CAD build for the part. Positions are in the model's coordinates, mm. A direction names the side the tool comes from. Coordinates: 2 decimals unless noted, no trailing zeros. Order: outer loops, then holes, each group sorted by start corner. A loop starts at its lowest first (then second) coordinate and runs counter-clockwise, first axis right, second up. Notation, with made-up numbers: (-20, 79) - (1, 79) arc R20 ccw to (1, 100) - close; hole circle Ø7 at (72, 74.25). An arc over 180 degrees is marked (long way). Return JSON: item names as keys, results as strings.
from build123d import *

# Parameters (mm, degrees)
EYE_PLATE_11MM_DEPTH    = 11
FLOOR_PLATE_11MM_DEPTH  = 11
SIDE_WALL_11MM_DEPTH    = 11
INCLINED_WEB_PROFILE_W  = 102
INCLINED_WEB_PROFILE_H  = 76
INCLINED_WEB_11MM_DEPTH = 11
END_CAP_PROFILE_W       = 35
END_CAP_PROFILE_H       = 76
END_CAP_16MM_DEPTH      = 16
PIVOT_BORE_PROFILE_R    = 19
PIVOT_BORE_38_DEPTH     = 11


with BuildPart() as part:
    # Eye Plate Profile → Eye Plate 11mm (new body)
    with BuildSketch(Plane.XY):
        with BuildLine():
            Line((0, 0), (113, 0))
            Line((113, 0), (113, 63))
            Line((113, 63), (25, 63))
            ThreePointArc((25, 63), (7.32233047, 55.67766953), (0, 38))
            Line((0, 38), (0, 0))
        make_face()
    extrude(amount=EYE_PLATE_11MM_DEPTH)

    # Floor Plate Profile → Floor Plate 11mm (add)
    with BuildSketch(Plane(origin=(113, 0, 0), x_dir=(0, 0, -1), z_dir=(1, 0, 0))):
        Polygon((0, 0), (76, 0), (76, 100), (0, 63), align=None)
    extrude(amount=-FLOOR_PLATE_11MM_DEPTH)

    # Side Wall Profile → Side Wall 11mm (add)
    with BuildSketch(Plane(origin=(0, 0, -76), x_dir=(-1, 0, 0), z_dir=(0, 0, -1))):
        Polygon((-113, 0), (0, 0), (0, 11), (-75, 100), (-113, 100), align=None)
    extrude(amount=SIDE_WALL_11MM_DEPTH)

    # Inclined Web Profile → Inclined Web 11mm (add)
    with BuildSketch(Plane.XZ):
        with Locations((51, -38)):
            Rectangle(INCLINED_WEB_PROFILE_W, INCLINED_WEB_PROFILE_H)
    extrude(amount=-INCLINED_WEB_11MM_DEPTH)

    # End Cap Profile → End Cap 16mm (add)
    with BuildSketch(Plane(origin=(0, 11, 0), x_dir=(1, 0, 0), z_dir=(0, 1, 0))):
        with Locations((84.5, 38)):
            Rectangle(END_CAP_PROFILE_W, END_CAP_PROFILE_H)
    extrude(amount=END_CAP_16MM_DEPTH)

    # Pivot Bore Profile → Pivot Bore Ø38 (cut)
    with BuildSketch(Plane.XY.offset(11)):
        with Locations((25, 38)):
            Circle(PIVOT_BORE_PROFILE_R)
    extrude(amount=-PIVOT_BORE_38_DEPTH, mode=Mode.SUBTRACT)


solid = part.part
Item 1: Band-saw the part on A-A, the plane x = 69. List the corners of the cut face in (y, z).
Findings below:
{"outline": "(0, -87) - (92.88, -87) - (92.88, -76) - (27, -76) - (27, 0) - (63, 0) - (63, 11) - (0, 11) - close"}
Item 2: Band-saw the part on D-D, the plane x = 17. List the corners of the cut face in (y, z).
Findings below:
{"outline": "(0, -87) - (31.17, -87) - (31.17, -76) - (11, -76) - (11, 0) - (20.77, 0) - (20.77, 11) - (0, 11) - close; (55.23, 0) - (61.69, 0) - (61.69, 11) - (55.23, 11) - close"}
Item 3: Mould opens along Z. For faces 1 (the flat face through (107.58, 81.76, -38.53)), 2 (the flat face through (67, 19, -37)), 3 (the flat face through (56, 0, -37)) say: released by +Z, released by -Z, zero draft, split by the parting line, or undercut.
Findings below:
{"face 1": "released by +Z", "face 2": "undercut", "face 3": "zero draft"}
Item 4: Band-saw the part on B-B, the plane y = 30. List the corners of the cut face in (x, z).
Findings below:
{"outline": "(0, 0) - (7.77, 0) - (7.77, 11) - (0, 11) - close; (16.01, -87) - (113, -87) - (113, 11) - (42.23, 11) - (42.23, 0) - (102, 0) - (102, -76) - (16.01, -76) - close"}
Item 5: Wall check: L1, parallel to Z at x = 77, y = 39; L2, parallel to Y at x = 25, z = 8; L3, parallel to Y at x = 88, z = -18. Give the ranges that are in metal, low to high. Write a range as [from, to].
Findings below:
{"L1": "z = [-87, -76], [0, 11]", "L2": "y = [0, 19], [57, 63]", "L3": "y = [0, 27]"}
Item 6: Drop flat-ended pins along their axis: P1, Ø5.5, axis at x = 58, z = 7.5, coming from the +Y side; P2, Ø17.5, axis at x = 88.5, z = -26.5, coming from the +Y side; P3, Ø4, axis at x = 33, y = 48, coming from the +Z side. Give the stop position or say it passes through.
Findings below:
{"P1": "stops at y = 63", "P2": "stops at y = 27", "P3": "stops at z = -76"}
Item 7: Band-saw the part on C-C, the plane z = 2. List the corners of the cut face in (x, y).
Findings below:
{"outline": "(0, 0) - (113, 0) - (113, 63) - (25, 63) arc R25 ccw to (0, 38) - close; hole circle Ø38 at (25, 38)"}
Item 8: Which spindle directions (+Z, -Z, +X, -X, +Y, -Y) get a long thin tool onto all of the face, cutting with end or side? Do faces 4 (the flat face through (70, 63, 5)), 5 (the cylindrical face through (20.881, 19.452, 5.577)), 6 (the flat face through (36.98, 54.88, -81.42)), 7 (the flat face through (63, 56, -76)). Say none if no direction does.
Findings below:
{"face 4": "+Z, +X, -X, +Y", "face 5": "+Z", "face 6": "-Z, -X, +Y", "face 7": "-X, +Y"}
